Read the model definition and answer for the solid it produces. Units are mm, in the model's axes. A direction names the side the tool comes from. Coordinates: 2 decimals unless noted, no trailing zeros. Loops run counter-clockwise (first coordinate to the right, second up) from the corner with the lowest first, then second, coordinate; pieces in that order, holes last. Notation, with made-up numbers: (18, 5) - (74, 5) arc R15 ccw to (74, 17) - close; hole circle Ø4 at (-29, -36). An arc over 180 degrees is marked (long way). Use CSV: the item, a comma, the result in double quotes.
```python
from build123d import *

# Parameters (mm, degrees)
BOSS_EXTRUDE1_DEPTH = 2300
LPATTERN1_COUNT     = 10
LPATTERN1_PITCH     = 230


with BuildPart() as part:
    # Sketch1 → Boss-Extrude1 (new body)
    with BuildSketch(Plane(origin=(0, 0, 0), x_dir=(1, 0, 0), z_dir=(0, 1, 0))):
        Polygon((-70, 10), (-70, 50), (70, 50), (70, 10), (110, 10), (110, -10), (-110, -10), (-110, 10), align=None)
    extrude(amount=BOSS_EXTRUDE1_DEPTH)

    # Sketch3 → Tap Drill for M10 Tap1 (revolve, cut)
    with BuildSketch(Plane(origin=(70, 2185, -30), x_dir=(0, 0, -1), z_dir=(0, 1, 0))):
        Polygon((0, 0), (0, 27.553657631), (4.25, 25), (4.25, 0.020977491), (4.275, 0), align=None)
    tap_drill_for_m10_tap1 = revolve(axis=Axis((76.35, 2185, -30), (-1, 0, 0)), mode=Mode.SUBTRACT)

    # LPattern1: Tap Drill for M10 Tap1 ×10
    with Locations(*[(0, -i * LPATTERN1_PITCH, 0) for i in range(1, LPATTERN1_COUNT)]):
        add(tap_drill_for_m10_tap1, mode=Mode.SUBTRACT)

    # Mirror1: Tap Drill for M10 Tap1 across plane
    add(tap_drill_for_m10_tap1.mirror(Plane(origin=(0, 0, 0), x_dir=(0, 0, 1), z_dir=(1, 0, 0))), mode=Mode.SUBTRACT)

    # Mirror1 copy 1 sketch → Mirror1 copy 1 (revolve, cut)
    with BuildSketch(Plane(origin=(-70, 1955, -30), x_dir=(0, 0, -1), z_dir=(0, 1, 0))):
        Polygon((0, 0), (0, -27.553657631), (4.25, -25), (4.25, -0.020977491), (4.275, 0), align=None)
    revolve(axis=Axis((-76.35, 1955, -30), (-1, 0, 0)), mode=Mode.SUBTRACT)

    # Mirror1 copy 2 sketch → Mirror1 copy 2 (revolve, cut)
    with BuildSketch(Plane(origin=(-70, 1725, -30), x_dir=(0, 0, -1), z_dir=(0, 1, 0))):
        Polygon((0, 0), (0, -27.553657631), (4.25, -25), (4.25, -0.020977491), (4.275, 0), align=None)
    revolve(axis=Axis((-76.35, 1725, -30), (-1, 0, 0)), mode=Mode.SUBTRACT)

    # Mirror1 copy 3 sketch → Mirror1 copy 3 (revolve, cut)
    with BuildSketch(Plane(origin=(-70, 1495, -30), x_dir=(0, 0, -1), z_dir=(0, 1, 0))):
        Polygon((0, 0), (0, -27.553657631), (4.25, -25), (4.25, -0.020977491), (4.275, 0), align=None)
    revolve(axis=Axis((-76.35, 1495, -30), (-1, 0, 0)), mode=Mode.SUBTRACT)

    # Mirror1 copy 4 sketch → Mirror1 copy 4 (revolve, cut)
    with BuildSketch(Plane(origin=(-70, 1265, -30), x_dir=(0, 0, -1), z_dir=(0, 1, 0))):
        Polygon((0, 0), (0, -27.553657631), (4.25, -25), (4.25, -0.020977491), (4.275, 0), align=None)
    revolve(axis=Axis((-76.35, 1265, -30), (-1, 0, 0)), mode=Mode.SUBTRACT)

    # Mirror1 copy 5 sketch → Mirror1 copy 5 (revolve, cut)
    with BuildSketch(Plane(origin=(-70, 1035, -30), x_dir=(0, 0, -1), z_dir=(0, 1, 0))):
        Polygon((0, 0), (0, -27.553657631), (4.25, -25), (4.25, -0.020977491), (4.275, 0), align=None)
    revolve(axis=Axis((-76.35, 1035, -30), (-1, 0, 0)), mode=Mode.SUBTRACT)

    # Mirror1 copy 6 sketch → Mirror1 copy 6 (revolve, cut)
    with BuildSketch(Plane(origin=(-70, 805, -30), x_dir=(0, 0, -1), z_dir=(0, 1, 0))):
        Polygon((0, 0), (0, -27.553657631), (4.25, -25), (4.25, -0.020977491), (4.275, 0), align=None)
    revolve(axis=Axis((-76.35, 805, -30), (-1, 0, 0)), mode=Mode.SUBTRACT)

    # Mirror1 copy 7 sketch → Mirror1 copy 7 (revolve, cut)
    with BuildSketch(Plane(origin=(-70, 575, -30), x_dir=(0, 0, -1), z_dir=(0, 1, 0))):
        Polygon((0, 0), (0, -27.553657631), (4.25, -25), (4.25, -0.020977491), (4.275, 0), align=None)
    revolve(axis=Axis((-76.35, 575, -30), (-1, 0, 0)), mode=Mode.SUBTRACT)

    # Mirror1 copy 8 sketch → Mirror1 copy 8 (revolve, cut)
    with BuildSketch(Plane(origin=(-70, 345, -30), x_dir=(0, 0, -1), z_dir=(0, 1, 0))):
        Polygon((0, 0), (0, -27.553657631), (4.25, -25), (4.25, -0.020977491), (4.275, 0), align=None)
    revolve(axis=Axis((-76.35, 345, -30), (-1, 0, 0)), mode=Mode.SUBTRACT)

    # Mirror1 copy 9 sketch → Mirror1 copy 9 (revolve, cut)
    with BuildSketch(Plane(origin=(-70, 115, -30), x_dir=(0, 0, -1), z_dir=(0, 1, 0))):
        Polygon((0, 0), (0, -27.553657631), (4.25, -25), (4.25, -0.020977491), (4.275, 0), align=None)
    revolve(axis=Axis((-76.35, 115, -30), (-1, 0, 0)), mode=Mode.SUBTRACT)


solid = part.part
```
Q1. Find the intervals of material crossed by probe 1 along Z at (x, y) = (56.25, 1495); probe 2 along X at (y, z) = (1695, -14.5); probe 3 along Z at (x, y) = (79, 2086.5), in increasing order. Write a range as [from, to].
Reported:
probe 1,"z = [-50, -34.25], [-25.75, 10]"
probe 2,"x = [-70, 70]"
probe 3,"z = [-10, 10]"
Q2. The part is cut by section A-A on y = 388. Determine the outline of the cut face in (x, z), and give its area (3 significant figures).
Reported:
outline,"(-110, -10) - (-70, -10) - (-70, -50) - (70, -50) - (70, -10) - (110, -10) - (110, 10) - (-110, 10) - close"
area,"10,000 mm²"
Q3. A tool of negligible diameter and unlimited length cuts with its end or side. For faces 1 (the face through (70, 1134, -30)), 2 (the face through (-1, 1134, -50)), 3 (the face through (-70, 1134, -30)), from which of +Z, -Z, +X, -X, +Y, -Y can it reach the whole face along a straight path? Write none if from no direction.
Reported:
face 1,"-Z, +X, +Y, -Y"
face 2,"-Z, +X, -X, +Y, -Y"
face 3,"-Z, -X, +Y, -Y"
Q4. Given P1, Ø7, axis at y = 2185, z = -30, coming from the -X side; P2, Ø12, axis at y = 2033.5, z = -23, coming from the +X side; P3, Ø5, axis at y = 115, z = -30, coming from the -X side, each flat-ended and moving along its own axis, determine where each tip first touches the part or whether it passes through.
Reported:
P1,"stops at x = -44.55"
P2,"stops at x = 70"
P3,"stops at x = -43.95"
